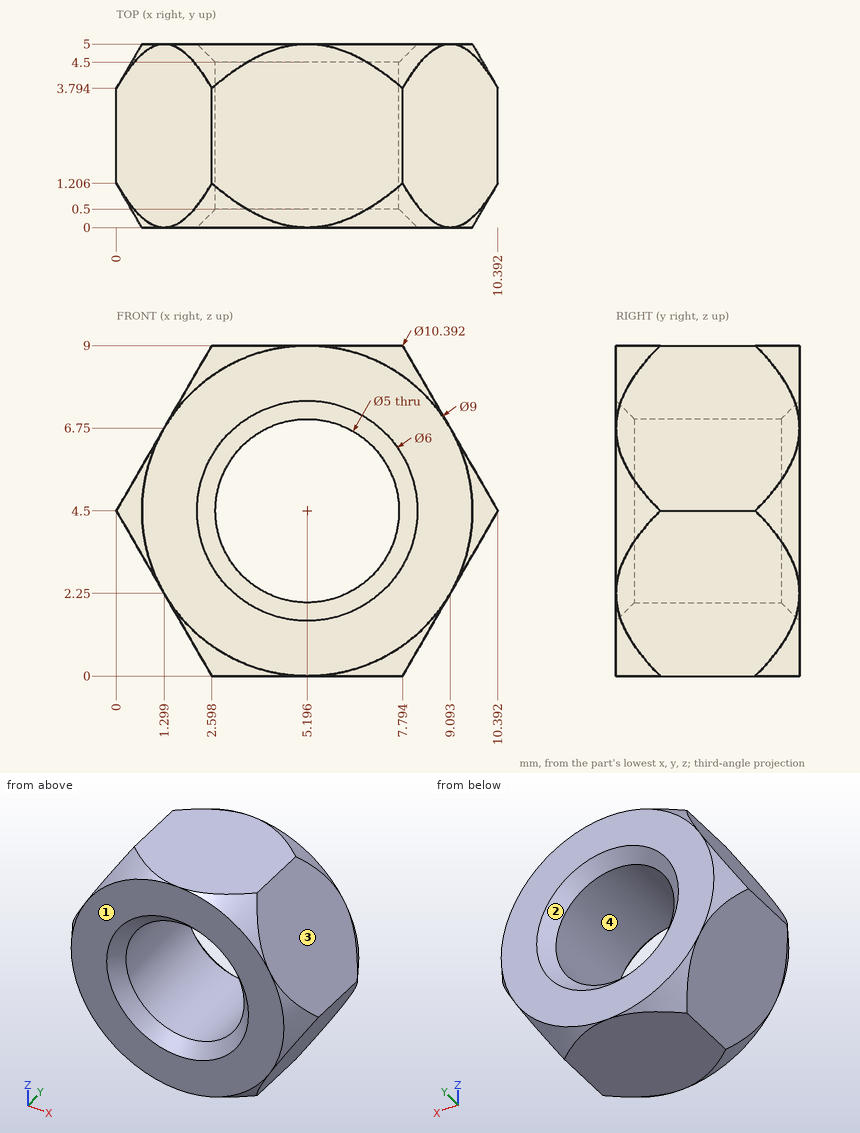
Study the drawing (mm; zero at the part's minimum x, y, z) and answer. Round coordinates to 2 decimals unless told otherwise and drop trailing zeros. Answer as CSV lines item,"result". Start each with the question number.
(1) Find the intervals of material crossed by probe 1 along Z at (x, y) = (5.5, 1); probe 2 along Z at (x, y) = (3.5, 3.3) (1 decimal); probe 3 along X at (y, z) = (1.1, 1), in increasing order.
(2) This flat-tipped pin is pushed along its axis until it touches: pin 1 (1 mm diameter, centred on y = 2.5, z = 1, fed in from -X). Where does it stop, or does it pass through?
(3) The mould has two halves that part along X. Classify the marked faces 1, 2, 3 and 4: +X half, -X half, draft (parallel to the pull), parting line (faces both ways), or undercut.
Output values:
1,probe 1,"z = 0 to 2.02, 6.98 to 9"
1,probe 2,"z = 0 to 2.7, 6.3 to 9"
1,probe 3,"x = 2.02 to 8.37"
2,pin 1,"stops at x = 1.73"
3,face 1,"draft"
3,face 2,"undercut"
3,face 3,"+X half"
3,face 4,"undercut"
